```python
from build123d import *

# Parameters (mm, degrees)
SKETCH_1_W                = 60
SKETCH_1_H                = 30
EXTRUDE_1_DEPTH           = 4
CHAMFER_1_SIZE            = 2
HOLE_WIZARD_1_D           = 4.5
HOLE_WIZARD_1_CBORE_D     = 8
HOLE_WIZARD_1_CBORE_DEPTH = 4.6
M10X1_0_1_D               = 9


with BuildPart() as part:
    # 草图1 → 凸台-拉伸1 (new, symmetric)
    with BuildSketch(Plane(origin=(0, 0, 0), x_dir=(1, 0, 0), z_dir=(0, 1, 0))):
        Rectangle(SKETCH_1_W, SKETCH_1_H)
    extrude(amount=EXTRUDE_1_DEPTH, both=True)

    # 倒角1
    chamfer_1_edges = [part.edges().sort_by_distance(p)[0] for p in [
        (30, 0, 15),
        (-30, 0, 15),
        (-30, 0, -15),
        (30, 0, -15),
    ]]
    chamfer(chamfer_1_edges, length=CHAMFER_1_SIZE)

    # 打孔尺寸(%根据)内六角圆柱头螺钉的类型1 (through all)
    with Locations(Plane(origin=(0, 4, 0), x_dir=(1, 0, 0), z_dir=(0, 1, 0))):
        with Locations((0, -10), (0, 10)):
            CounterBoreHole(HOLE_WIZARD_1_D / 2, HOLE_WIZARD_1_CBORE_D / 2, HOLE_WIZARD_1_CBORE_DEPTH)

    # M10x1.0 螺纹孔1 (through all)
    with Locations(Plane(origin=(0, -4, 0), x_dir=(-1, 0, 0), z_dir=(0, -1, 0))):
        with Locations((-22.5, 0), (22.5, 0)):
            Hole(M10X1_0_1_D / 2)


solid = part.part
```
Design review of the part built by this model. Coordinates are the model's own, in mm. A direction names the side the tool comes from. Give positions to 0.01 mm unless a question says otherwise; leave off trailing zeros. Write each loop counter-clockwise with the first axis right and the second up, starting at its lowest first coordinate (ties: lowest second). Pieces come first, ordered by that corner, then holes. Notation, with made-up numbers: (-16.5, 27.5) - (-9.5, 27.5) arc R28 cw to (-9.5, 47.5) - close; hole circle Ø3 at (42, 23). An arc over 180 degrees is marked (long way). Return JSON: item names as keys, results as strings. Group by question number.
(1) We need section D-D, the plane z = 0. Give the boundary of the cut face in (x, y), then the cut area to 3 significant figures.
(2) Insertion check: pin 1 (4 mm diameter, centred on x = 0, z = -10, fed in from +Y); pin 2 (5 mm diameter, centred on x = 0, z = 10, fed in from +Y). Each pin has a flat end and moves straight along its axis. Give the tip position at first contact, or say it passes through.
(3) We need section A-A, the plane x = 22.5. Give the boundary of the cut face in (y, z), then the cut area to 3 significant figures.
(4) We need section B-B, the plane z = -10. Give the boundary of the cut face in (x, y), then the cut area to 3 significant figures.
(5) Mouldability with a two-part tool opening along Z and no side actions: class faces 1 (the flat face through (0, -4, 0)), 2 (the flat face through (0, 0, -15)), 3 (the cylindrical face through (18, 0, 0)) as +Z half, -Z half, draft (parallel to the pull), parting line (faces both ways), or undercut.
(6) To check wall thickness, follow probe 1 along Z at (x, y) = (0, -3.3); probe 2 along X at (y, z) = (-3.2, 10); probe 3 along Z at (x, y) = (22.5, 1.25). State the ranges of each line that lie inside material, in increasing order.
(7) We need section C-C, the plane y = -3. Give the boundary of the cut face in (x, z).
(8) Machinability: for faces 4 (the flat face through (0, 4, 0)), 5 (the flat face through (2, -0.6, 12)), which of the approach directions +Z, -Z, +X, -X, +Y, -Y give a long, thin tool a straight path to every point of the face, cutting with its end or side? Answer none if there is none.
Reported:
{
 "1": {"outline": "(-30, -4) - (-27, -4) - (-27, 4) - (-30, 4) - close; (-18, -4) - (18, -4) - (18, 4) - (-18, 4) - close; (27, -4) - (30, -4) - (30, 4) - (27, 4) - close", "area": "336 mm2"},
 "2": {"pin 1": "passes through", "pin 2": "stops at y = -0.6"},
 "3": {"outline": "(-4, -15) - (4, -15) - (4, -4.5) - (-4, -4.5) - close; (-4, 4.5) - (4, 4.5) - (4, 15) - (-4, 15) - close", "area": "168 mm2"},
 "4": {"outline": "(-30, -4) - (-2.25, -4) - (-2.25, -0.6) - (-4, -0.6) - (-4, 4) - (-30, 4) - close; (2.25, -4) - (30, -4) - (30, 4) - (4, 4) - (4, -0.6) - (2.25, -0.6) - close", "area": "428 mm2"},
 "5": {"face 1": "draft", "face 2": "-Z half", "face 3": "undercut"},
 "6": {"probe 1": "z = -15 to -12.25, -7.75 to 7.75, 12.25 to 15", "probe 2": "x = -30 to -2.25, 2.25 to 30", "probe 3": "z = -15 to -4.5, 4.5 to 15"},
 "7": {"outline": "(-30, -13) - (-28, -15) - (28, -15) - (30, -13) - (30, 13) - (28, 15) - (-28, 15) - (-30, 13) - close; hole circle Ø9 at (-22.5, 0); hole circle Ø4.5 at (0, -10); hole circle Ø4.5 at (0, 10); hole circle Ø9 at (22.5, 0)"},
 "8": {"face 4": "+Z, -Z, +X, -X, +Y", "face 5": "+Y"}
}
